```python
from build123d import *

# Parameters (mm, degrees)
SKETCH1_R           = 2.5765
SKETCH1_R_2         = 2.4585
BOSS_EXTRUDE1_DEPTH = 19
SKETCH2_R           = 4
SKETCH2_R_2         = 3.3235
SKETCH2_R_3         = 1.2995
CUT_EXTRUDE1_DEPTH  = 81.907354425
SKETCH3_R           = 5
CUT_EXTRUDE2_DEPTH  = 5


with BuildPart() as part:
    # Sketch1 → Boss-Extrude1 (new body)
    with BuildSketch(Plane.XY):
        with BuildLine():
            Line((0, 0), (25.5415, 0))
            ThreePointArc((25.5415, 0), (28, 2.4585), (30.4585, 0))
            Line((30.4585, 0), (33.63748457, 0))
            Line((33.63748457, 0), (33.63748457, -7.90741809))
            Line((33.63748457, -7.90741809), (77, -7.90741809))
            Line((77, -7.90741809), (77, 8.09258191))
            Line((77, 8.09258191), (0, 8.09258191))
            Line((0, 8.09258191), (0, 0))
        make_face()
        with Locations((59, 0.09258191)):
            Circle(SKETCH1_R, mode=Mode.SUBTRACT)
        with Locations((44, 0.09258191)):
            Circle(SKETCH1_R_2, mode=Mode.SUBTRACT)
    extrude(amount=BOSS_EXTRUDE1_DEPTH)

    # Sketch2 → Cut-Extrude1 (cut, through all)
    with BuildSketch(Plane(origin=(0, 8.09258191, 0), x_dir=(1, 0, 0), z_dir=(0, 1, 0))):
        with Locations(Location((67, -9.5, 0), (0, 0, 180))):
            Circle(SKETCH2_R)
        with Locations(Location((52, -9.5, 0), (0, 0, 180))):
            Circle(SKETCH2_R_2)
        with Locations(Location((37, -9.5, 0), (0, 0, 180))):
            Circle(SKETCH2_R)
        with Locations(Location((13.50002, -9.5, 0), (0, 0, 180))):
            Circle(SKETCH2_R_3)
    extrude(amount=-CUT_EXTRUDE1_DEPTH, mode=Mode.SUBTRACT)

    # Sketch3 → Cut-Extrude2 (cut)
    with BuildSketch(Plane(origin=(0, 0, 0), x_dir=(-1, 0, 0), z_dir=(0, -1, 0))):
        with Locations(Location((-13.50002, -9.5, 0), (0, 0, 90))):
            Circle(SKETCH3_R)
    extrude(amount=-CUT_EXTRUDE2_DEPTH, mode=Mode.SUBTRACT)


solid = part.part
```
Verification items for the finished model (mm, model axes). A direction names the side the tool comes from. Coordinates: 2 decimals unless noted, no trailing zeros. Loops run counter-clockwise (first coordinate to the right, second up) from the corner with the lowest first, then second, coordinate; pieces in that order, holes last. Notation, with made-up numbers: (-9.75, -14) -> (8.25, -14) arc R19 cw to (8.25, 6) -> close; hole circle Ø7 at (45.25, 24). An arc over 180 degrees is marked (long way). Answer in a Markdown table with one row per item.
1) Depth check by flat-ended pin: P1, Ø10, axis at x = 66, z = 8.5, coming from the +Y side; P2, Ø3, axis at x = 16.5, z = 6, coming from the -Y side; P3, Ø5, axis at x = 13.5, z = 11, coming from the -Y side; P4, Ø8, axis at y = -6, z = 4, coming from the -X side. Enter the tip coordinate at first touch or a pass-through.
The answers:
| item | result |
|---|---|
| P1 | stops at y = 8.09 |
| P2 | stops at y = 0 |
| P3 | stops at y = 5 |
| P4 | stops at x = 33.64 |
2) Section check B-B (y = 5.75). Record the cut outline in (x, z).
The answers:
| item | result |
|---|---|
| outline | (0, 0) -> (77, 0) -> (77, 19) -> (0, 19) -> close; hole circle Ø2.6 at (13.5, 9.5); hole circle Ø8 at (37, 9.5); hole circle Ø6.65 at (52, 9.5); hole circle Ø8 at (67, 9.5) |
3) Section check D-D (y = -5.25). Record the cut outline in (x, z).
The answers:
| item | result |
|---|---|
| outline | (33.64, 0) -> (77, 0) -> (77, 19) -> (33.64, 19) -> (33.64, 11.67) arc R4 cw (long way) to (33.64, 7.33) -> close; hole circle Ø6.65 at (52, 9.5); hole circle Ø8 at (67, 9.5) |
4) Section check A-A (x = 59). Record the cut outline in (y, z), and give its area (3 significant figures).
The answers:
| item | result |
|---|---|
| outline | (-7.91, 0) -> (-2.48, 0) -> (-2.48, 19) -> (-7.91, 19) -> close; (2.67, 0) -> (8.09, 0) -> (8.09, 19) -> (2.67, 19) -> close |
| area | 206 mm2 |
5) Draft check along X on faces 1 (the face through (0, 4, 9)), 2 (the face through (47, 2, 19)), 3 (the face through (27.946, 2.458, 9.367)). Enter one of: released by +X, released by -X, zero draft, split by the parting line, or undercut.
The answers:
| item | result |
|---|---|
| face 1 | released by -X |
| face 2 | zero draft |
| face 3 | undercut |
6) Section check C-C (z = 9.5). Record the cut outline in (x, y).
The answers:
| item | result |
|---|---|
| outline | (0, 0) -> (8.5, 0) -> (8.5, 5) -> (12.2, 5) -> (12.2, 8.09) -> (0, 8.09) -> close; (14.8, 5) -> (18.5, 5) -> (18.5, 0) -> (25.54, 0) arc R2.46 cw to (30.46, 0) -> (33, 0) -> (33, 8.09) -> (14.8, 8.09) -> close; (41, -7.91) -> (48.68, -7.91) -> (48.68, 8.09) -> (41, 8.09) -> close; (55.32, -7.91) -> (63, -7.91) -> (63, 8.09) -> (55.32, 8.09) -> close; (71, -7.91) -> (77, -7.91) -> (77, 8.09) -> (71, 8.09) -> close; hole circle Ø4.92 at (44, 0.09); hole circle Ø5.15 at (59, 0.09) |
7) Scan lines: line 1 along X through (y, z) = (0.25, 18); line 2 along Y through (x, z) = (44, 13.5); line 3 along X through (y, z) = (-2.75, 7.5). Record each from-to range of solid material in increasing order. Write a range as from..to.
The answers:
| item | result |
|---|---|
| line 1 | x = 0..25.55, 30.45..41.55, 46.45..56.43, 61.57..77 |
| line 2 | y = -7.91..-2.37, 2.55..8.09 |
| line 3 | x = 40.46..49.35, 54.65..63.54, 70.46..77 |
8) Access from +Z, -Z, +X, -X, +Y, -Y to the whole of each face (thin tool, end or side, straight path). Record for faces 4 (the face through (15, 2.46, 4.73)), 5 (the face through (46.27, -0.85, 9.37)), 6 (the face through (10, 0, 5)).
The answers:
| item | result |
|---|---|
| face 4 | -Y |
| face 5 | +Z, -Z |
| face 6 | +Z, -Z, -X, -Y |
